from build123d import *

# Parameters (mm, degrees)
SKETCH_2_R      = 55
EXTRUDE_1_DEPTH = 15
EXTRUDE_2_DEPTH = 25


with BuildPart() as part:
    # 草图1 → 旋转1 (revolve)
    with BuildSketch(Plane(origin=(0, 0, 0), x_dir=(1, 0, 0), z_dir=(0, 1, 0))):
        Polygon((0, 40), (-10, 40), (-10, -108), (-25, -108), (-55, -123), (0, -123), align=None)
    revolve(axis=Axis((0, 0, -40), (0, 0, 1)))

    # 草图2 → 凸台-拉伸1 (add)
    with BuildSketch(Plane.XY.offset(123)):
        Circle(SKETCH_2_R)
    extrude(amount=EXTRUDE_1_DEPTH)

    # 草图3 → 凸台-拉伸2 (add)
    with BuildSketch(Plane(origin=(0, 0, 108), x_dir=(-1, 0, 0), z_dir=(0, 0, -1))):
        Polygon((15, 25.980762114), (-15, 25.980762114), (-30, 0), (-15, -25.980762114), (15, -25.980762114), (30, 0), align=None)
    extrude(amount=EXTRUDE_2_DEPTH)


solid = part.part
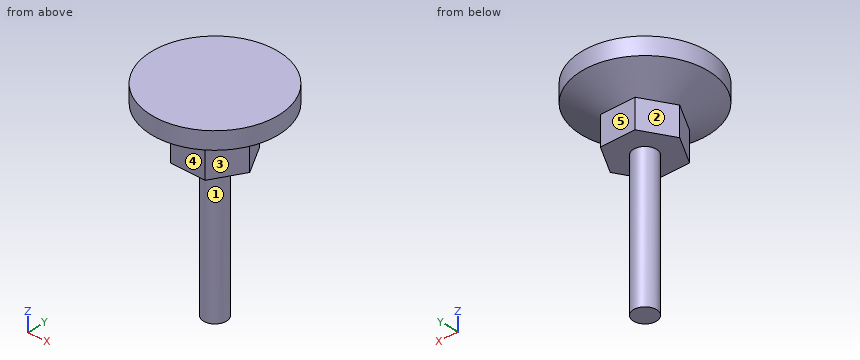
Source: CAD feature listing. Evaluate the final solid. Frame: model axes, mm. Face numbers are marked on the shaded views. A direction names the side the tool comes from. Round coordinates to 2 decimals unless told otherwise and drop trailing zeros. Loops run counter-clockwise (first coordinate to the right, second up) from the corner with the lowest first, then second, coordinate; pieces in that order, holes last. Notation, with made-up numbers: (67, -39) -> (117, -39) arc R7 cw to (117, -26) -> close; hole circle Ø8 at (53.5, -26.75). An arc over 180 degrees is marked (long way). Answer as a JSON object with one key per item and string values. Group by question number.
Q1. Section query B-B (z = 110). Output: boundary loops of the cut face in (x, y).
Q2. Ray query, line 1 (Z direction, x = -46.5, y = -6.5); line 2 (Z direction, x = 29, y = -42); line 3 (Y direction, x = -6.5, z = -13). Return the intervals inside material, ascending. Write a range as from..to.
Q3. Access query for the marked faces 1, 2, 3, 4 and 5. Directions: +Z, -Z, +X, -X, +Y, -Y. A direction counts if a zero-diameter tool reaches every point of the face in a straight line with its end or side. Return the directions, or none.
Q4. Section query A-A (x = 0). Output: boundary loops of the cut face in (y, z).
Q5. Contact query for flat-ended pins moving along their axis: P1, Ø8, axis at y = -2, z = 85, coming from the -X side; P2, Ø1, axis at x = -17.5, y = -13.5, coming from the -Z side; P3, Ø3, axis at y = 9.5, z = 40, coming from the -X side. Output: stop coordinate, or through.
Q6. Section query C-C (z = 60). Output: boundary loops of the cut face in (x, y), plus the area to 3 significant figures.
Completed:
{
 "1": {"outline": "circle Ø58 at (0, 0)"},
 "2": {"line 1": "118.98..138", "line 2": "121.02..138", "line 3": "-7.6..7.6"},
 "3": {"face 1": "-Z", "face 2": "-Z, -X, +Y", "face 3": "-Z, +X, -Y", "face 4": "-Z, +X, -X, -Y", "face 5": "-Z, +X, -X, +Y"},
 "4": {"outline": "(-55, 123) -> (-25, 108) -> (-25.98, 108) -> (-25.98, 83) -> (-10, 83) -> (-10, -40) -> (10, -40) -> (10, 83) -> (25.98, 83) -> (25.98, 108) -> (25, 108) -> (55, 123) -> (55, 138) -> (-55, 138) -> close"},
 "5": {"P1": "x = -30", "P2": "z = 83", "P3": "x = -6"},
 "6": {"outline": "circle Ø20 at (0, 0)", "area": "314 mm²"}
}
